Here's how the part is built. I have some questions about the finished solid (model axes, mm). Face numbers are marked on the shaded views. A direction names the side the tool comes from. Coordinates: 2 decimals unless noted, no trailing zeros. Order: outer loops, then holes, each group sorted by start corner. A loop starts at its lowest first (then second) coordinate and runs counter-clockwise, first axis right, second up. Notation, with made-up numbers: M -23.75,-29.5 L 26.25,-29.5 A13 ccw 26.25,-4.5 Z; hole C 19,45 d9. An arc over 180 degrees is marked long. One line per question, with ' | ' between items. Start each with the question number.
```python
from build123d import *

# Parameters (mm, degrees)
BOSS_EXTRUDE1_DEPTH = 30
SKETCH3_R           = 5
CUT_EXTRUDE1_DEPTH  = 3


with BuildPart() as part:
    # Sketch2 → Boss-Extrude1 (new body)
    with BuildSketch(Plane.XY):
        with BuildLine():
            Line((0, 0), (0, 30))
            Line((0, 30), (1, 30))
            ThreePointArc((1, 30), (2.414213562, 29.414213562), (3, 28))
            Line((3, 28), (3, 5))
            ThreePointArc((3, 5), (3.585786438, 3.585786438), (5, 3))
            Line((5, 3), (28, 3))
            ThreePointArc((28, 3), (29.414213562, 2.414213562), (30, 1))
            Line((30, 1), (30, 0))
            Line((30, 0), (0, 0))
        make_face()
    extrude(amount=BOSS_EXTRUDE1_DEPTH)

    # Sketch3 → Cut-Extrude1 (cut)
    with BuildSketch(Plane(origin=(0, 3, 0), x_dir=(1, 0, 0), z_dir=(0, 1, 0))):
        with Locations(Location((22, -15, 0), (0, 0, 270))):
            Circle(SKETCH3_R)
    extrude(amount=-CUT_EXTRUDE1_DEPTH, mode=Mode.SUBTRACT)


solid = part.part
```
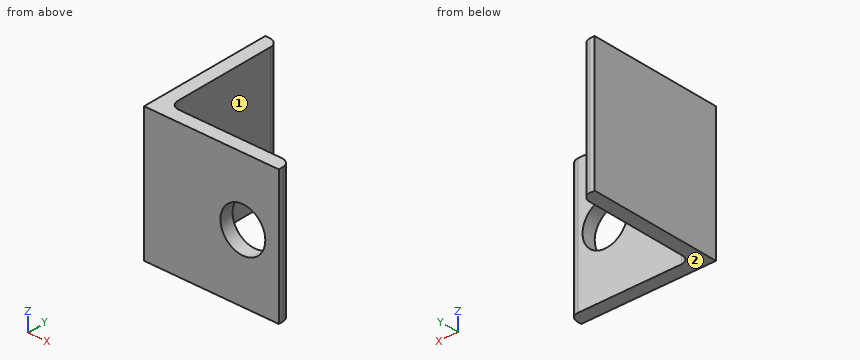
1. Will these pins go through, and if not, where does the flat tip stop? pin 1 (1.5 mm diameter, centred on x = 21, y = 5, fed in from -Z); pin 2 (10 mm diameter, centred on y = 7, z = 10.5, fed in from +X); pin 3 (11.5 mm diameter, centred on x = 22, z = 15, fed in from +Y).
2. I need wall thicknesses on line 1 (X direction, y = 1.05, z = 15); line 2 (Y direction, x = 14, z = 5.75). Which ranges of each line are inside material? Lowest first, please.
3. Imagine slicing it at D-D (x = 22). List the corners of the cut face in (y, z) for me, then the cut area to 3 significant figures.
4. Imagine slicing it at A-A (x = 26). List the corners of the cut face in (y, z) for me, then the cut area to 3 significant figures.
5. Imagine slicing it at B-B (z = 15). List the corners of the cut face in (x, y) for me, then the cut area to 3 significant figures.
6. Which directions (+Z, -Z, +X, -X, +Y, -Y) give clear straight access to the entire face, cutting with the end or side of a thin tool? Please do the marked faces 1 and 2.
7. Imagine slicing it at C-C (z = 23.25). List the corners of the cut face in (x, y) for me, then the cut area to 3 significant figures.
Entries:
1) pin 1: through | pin 2: x = 29.73 | pin 3: y = 3
2) line 1: 0 to 17, 27 to 30 | line 2: 0 to 3
3) outline: M 0,0 L 3,0 L 3,10 L 0,10 Z; M 0,20 L 3,20 L 3,30 L 0,30 Z | area: 60.0 mm²
4) outline: M 0,0 L 3,0 L 3,12 L 0,12 Z; M 0,18 L 3,18 L 3,30 L 0,30 Z | area: 72.0 mm²
5) outline: M 0,0 L 17,0 L 17,3 L 5,3 A2 cw 3,5 L 3,28 A2 ccw 1,30 L 0,30 Z; M 27,0 L 30,0 L 30,1 A2 ccw 28,3 L 27,3 Z | area: 140 mm²
6) face 1: +Z, -Z, +X, +Y | face 2: -Z, +X, -X, +Y, -Y
7) outline: M 0,0 L 30,0 L 30,1 A2 ccw 28,3 L 5,3 A2 cw 3,5 L 3,28 A2 ccw 1,30 L 0,30 Z | area: 170 mm²
